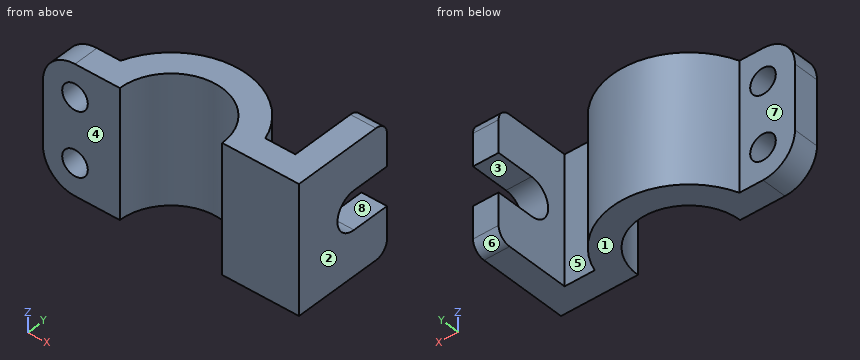
from build123d import *

# Parameters (mm, degrees)
ARCH_BODY_DEPTH             = 50
SIDE_RELIEF_CUT_DEPTH       = 50
END_RELIEF_CUT_DEPTH        = 50
ARCH_BORE_CUT_DEPTH         = 50
LUG_BLOCK_DEPTH             = 50
LUG_U_SLOT_DEPTH            = 50
FLANGE_BOLT_HOLES_PROFILE_R = 5
FLANGE_BOLT_HOLES_DEPTH     = 50


with BuildPart() as part:
    # Arch Body Profile → Arch Body (new body)
    with BuildSketch(Plane.XY):
        Polygon((0, 0), (100, 0), (100, 40), (90, 40), (90, 10), (0, 10), align=None)
    extrude(amount=ARCH_BODY_DEPTH)

    # Side Relief Profile → Side Relief Cut (cut)
    with BuildSketch(Plane(origin=(100, 0, 0), x_dir=(0, 0, -1), z_dir=(1, 0, 0))):
        with BuildLine():
            Line((-50, 40), (-50, 35))
            ThreePointArc((-50, 35), (-48.535533906, 38.535533906), (-45, 40))
            Line((-45, 40), (-50, 40))
        make_face()
        with BuildLine():
            Line((0, 40), (0, 35))
            ThreePointArc((0, 35), (-1.464466094, 38.535533906), (-5, 40))
            Line((-5, 40), (0, 40))
        make_face()
    extrude(amount=-SIDE_RELIEF_CUT_DEPTH, mode=Mode.SUBTRACT)

    # End Relief Profile → End Relief Cut (cut)
    with BuildSketch(Plane(origin=(100, 0, 0), x_dir=(0, 0, -1), z_dir=(1, 0, 0))):
        with BuildLine():
            Line((-17.5, 40), (-25, 40))
            Line((-25, 40), (-32.5, 40))
            Line((-32.5, 40), (-32.5, 25))
            ThreePointArc((-32.5, 25), (-25, 17.5), (-17.5, 25))
            Line((-17.5, 25), (-17.5, 40))
        make_face()
    extrude(amount=-END_RELIEF_CUT_DEPTH, mode=Mode.SUBTRACT)

    # Arch Bore Profile → Arch Bore Cut (cut)
    with BuildSketch(Plane(origin=(0, 10, 0), x_dir=(1, 0, 0), z_dir=(0, 1, 0))):
        with BuildLine():
            Line((0, -50), (12.5, -50))
            ThreePointArc((12.5, -50), (3.661165235, -46.338834765), (0, -37.5))
            Line((0, -37.5), (0, -50))
        make_face()
        with BuildLine():
            Line((0, 0), (12.5, 0))
            ThreePointArc((12.5, 0), (3.661165235, -3.661165235), (0, -12.5))
            Line((0, -12.5), (0, 0))
        make_face()
    extrude(amount=-ARCH_BORE_CUT_DEPTH, mode=Mode.SUBTRACT)

    # Lug Block Profile → Lug Block (add)
    with BuildSketch(Plane.XY.offset(50)):
        with BuildLine():
            Line((21.715728753, 10), (78.284271247, 10))
            ThreePointArc((78.284271247, 10), (50, 30), (21.715728753, 10))
        make_face()
    extrude(amount=-LUG_BLOCK_DEPTH)

    # Lug U-Slot Profile → Lug U-Slot (cut)
    with BuildSketch(Plane.XY.offset(50)):
        with BuildLine():
            Line((30, 0), (70, 0))
            ThreePointArc((70, 0), (50, 20), (30, 0))
        make_face()
    extrude(amount=-LUG_U_SLOT_DEPTH, mode=Mode.SUBTRACT)

    # Flange Bolt Holes Profile → Flange Bolt Holes (cut)
    with BuildSketch(Plane(origin=(0, 10, 0), x_dir=(1, 0, 0), z_dir=(0, 1, 0))):
        with Locations(Location((12.5, -37.5, 0), (0, 0, 270))):
            Circle(FLANGE_BOLT_HOLES_PROFILE_R)
        with Locations(Location((12.5, -12.5, 0), (0, 0, 270))):
            Circle(FLANGE_BOLT_HOLES_PROFILE_R)
    extrude(amount=-FLANGE_BOLT_HOLES_DEPTH, mode=Mode.SUBTRACT)


solid = part.part
Geometry: final body of the model. Coordinates: model frame, mm. Face numbers are marked on the shaded views. A direction names the side the tool comes from. Give positions to 0.01 mm unless a question says otherwise; leave off trailing zeros. Write each loop counter-clockwise with the first axis right and the second up, starting at its lowest first coordinate (ties: lowest second). Pieces come first, ordered by that corner, then holes.
(1) Cut plane C-C, the plane x = 11.5. Return loops of the section in (y, z).
(2) First-contact query: P1, Ø3.5, axis at x = 86.5, z = 27, coming from the +Y side; P2, Ø16, axis at x = 12.5, z = 12.5, coming from the -Y side; P3, Ø10, axis at y = 19.5, z = 6.5, coming from the -X side. Flat tips, straight axial feed; report the tip coordinate or a pass-through.
(3) Cut plane A-A, the plane y = 36.5. Return loops of the section in (x, z).
(4) Cut plane B-B, the plane z = 41. Return loops of the section in (x, y).
(5) Mould query, pull axis Z, two halves, no side actions, for the marked faces 1, 2 and 3. Classes: released by +Z, released by -Z, zero draft, split by the parting line, or undercut.
(6) Ray query, line 1 (X direction, y = 3, z = 12); line 2 (Z direction, x = 12, y = 6); line 3 (X direction, y = 5.25, z = 37.5). Return the intervals inside material, ascending.
(7) Access query for the marked faces 4, 5, 6, 7 and 8. Directions: +Z, -Z, +X, -X, +Y, -Y. A direction counts if a zero-diameter tool reaches every point of the face in a straight line with its end or side. Return the directions, or none.
(8) Cut plane D-D, the plane y = 31.5. Return loops of the section in (x, z).
Values follow:
1. outline: (0, 0.04) - (10, 0.04) - (10, 7.6) - (0, 7.6) - close; (0, 17.4) - (10, 17.4) - (10, 32.6) - (0, 32.6) - close; (0, 42.4) - (10, 42.4) - (10, 49.96) - (0, 49.96) - close
2. P1: stops at y = 10
2. P2: stops at y = 0
2. P3: stops at x = 23.74
3. outline: (90, 0.23) - (100, 0.23) - (100, 17.5) - (90, 17.5) - close; (90, 32.5) - (100, 32.5) - (100, 49.77) - (90, 49.77) - close
4. outline: (0.5, 0) - (8.93, 0) - (8.93, 10) - (0.5, 10) - close; (16.07, 0) - (30, 0) arc R20 cw to (70, 0) - (100, 0) - (100, 40) - (90, 40) - (90, 10) - (78.28, 10) arc R30 ccw to (21.72, 10) - (16.07, 10) - close
5. face 1: released by -Z
5. face 2: zero draft
5. face 3: undercut
6. line 1: x = 0.01 to 7.53, 17.47 to 30.23, 69.77 to 100
6. line 2: z = 0.01 to 7.53, 17.47 to 32.53, 42.47 to 49.99
6. line 3: x = 0 to 7.5, 17.5 to 30.7, 69.3 to 100
7. face 4: +Z, -Z, +X, -X, -Y
7. face 5: +Z, -Z, +Y
7. face 6: -Z, +X, -X, +Y
7. face 7: +Z, -Z, -X, +Y
7. face 8: +X, +Y
8. outline: (90, 0) - (100, 0) - (100, 17.5) - (90, 17.5) - close; (90, 32.5) - (100, 32.5) - (100, 50) - (90, 50) - close
